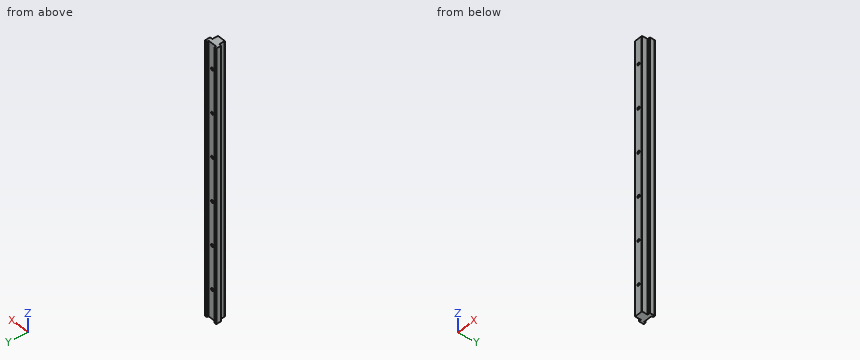
from build123d import *

# Parameters (mm, degrees)
BOSS_EXTRUDE1_DEPTH = 125
M3_TAPPED_HOLE1_D   = 2.5
CHAMFER1_SIZE       = 0.2
LPATTERN1_COUNT     = 6
LPATTERN1_PITCH     = 40


with BuildPart() as part:
    # Sketch1 → Boss-Extrude1 (new, symmetric)
    with BuildSketch(Plane.XY):
        Polygon((4, 0), (-4, 0), (-4, 1.5), (-6, 1.5), (-6, -3.2), (-3.7, -3.2), (-3.7, -8.5), (3.7, -8.5), (3.7, -3.2), (6, -3.2), (6, 1.5), (4, 1.5), align=None)
    extrude(amount=BOSS_EXTRUDE1_DEPTH, both=True)

    # M3 Tapped Hole1 (through all)
    with Locations(Plane(origin=(0, 0, 0), x_dir=(1, 0, 0), z_dir=(0, 1, 0))):
        with Locations((0, 98.25)):
            m3_tapped_hole1 = Hole(M3_TAPPED_HOLE1_D / 2)

    # Chamfer1
    chamfer1_edges = [part.edges().sort_by_distance(p)[0] for p in [
        (4, 1.5, 0),
        (6, 1.5, 0),
        (6, -3.2, 0),
        (3.7, -8.5, 0),
        (-3.7, -8.5, 0),
        (-6, -3.2, 0),
        (-6, 1.5, 0),
        (-4, 1.5, 0),
    ]]
    chamfer(chamfer1_edges, length=CHAMFER1_SIZE)

    # LPattern1: M3 Tapped Hole1 ×6
    with Locations(*[(0, 0, i * LPATTERN1_PITCH) for i in range(1, LPATTERN1_COUNT)]):
        add(m3_tapped_hole1, mode=Mode.SUBTRACT)


solid = part.part
Model file for the job. Use its own axes, mm. Give positions to 0.01 mm unless a question says otherwise; leave off trailing zeros. Loops run counter-clockwise (first coordinate to the right, second up) from the corner with the lowest first, then second, coordinate; pieces in that order, holes last.
1) Flat gauge pins, fed straight in: pin 1 Ø6.5 at (x, z) = (2, 6) entering from +Y; pin 2 Ø1 at (y, z) = (-6.5, -16.5) entering from -X; pin 3 Ø1 at (x, z) = (5, 34.5) entering from -Y; pin 4 Ø2.5 at (y, z) = (-6, 19) entering from +X. Where does each tip first touch, or does it go through?
2) Saw through at B-B (y = -6). Write the cut outline in (x, z), plus the area to 3 significant figures.
3) Saw through at A-A (z = 70). Write the cut outline in (x, y), plus the area to 3 significant figures.
4) Wall check: line 1 (X direction, y = -3, z = -98.25); line 2 (X direction, y = 1, z = 7.5); line 3 (Y direction, x = 4.25, z = 45). Give the ranges that are in metal, low to high.
Answer block:
1. pin 1: stops at y = 1.5
1. pin 2: stops at x = -3.7
1. pin 3: stops at y = -3.2
1. pin 4: stops at x = 3.7
2. outline: (-3.7, -125) - (3.7, -125) - (3.7, 125) - (-3.7, 125) - close; hole circle Ø2.5 at (0, -98.25); hole circle Ø2.5 at (0, -58.25); hole circle Ø2.5 at (0, -18.25); hole circle Ø2.5 at (0, 21.75); hole circle Ø2.5 at (0, 61.75); hole circle Ø2.5 at (0, 101.75)
2. area: 1,820 mm2
3. outline: (-6, -3) - (-5.8, -3.2) - (-3.7, -3.2) - (-3.7, -8.3) - (-3.5, -8.5) - (3.5, -8.5) - (3.7, -8.3) - (3.7, -3.2) - (5.8, -3.2) - (6, -3) - (6, 1.3) - (5.8, 1.5) - (4.2, 1.5) - (4, 1.3) - (4, 0) - (-4, 0) - (-4, 1.3) - (-4.2, 1.5) - (-5.8, 1.5) - (-6, 1.3) - close
3. area: 83.5 mm2
4. line 1: x = -6 to -1.25, 1.25 to 6
4. line 2: x = -6 to -4, 4 to 6
4. line 3: y = -3.2 to 1.5
